from build123d import *

# Parameters (mm, degrees)
CHAMFER1_SIZE  = 3
CHAMFER1_SIZE2 = 0.803847577


with BuildPart() as part:
    # Sketch1 → Revolve1 (revolve)
    with BuildSketch(Plane.XY, mode=Mode.PRIVATE) as revolve1_sk:
        Polygon((42.5, 31), (50, 31), (50, 3), (63.5, 3), (63.5, 0), (67.5, 0), (67.5, -8), (42.5, -8), align=None)
    revolve(revolve1_sk.sketch.rotate(Axis((0, 0, 0), (0, 1, 0)), 90), axis=Axis((0, 0, 0), (0, 1, 0)))

    # Chamfer1
    chamfer1_edges = [part.edges().sort_by_distance(p)[0] for p in [
        (0, 31, 50),
    ]]
    chamfer1_side = [part.faces().sort_by_distance(p)[0] for p in [
        (0, 17, 50),
    ]]
    chamfer(chamfer1_edges, length=CHAMFER1_SIZE, length2=CHAMFER1_SIZE2, reference=chamfer1_side[0])


solid = part.part
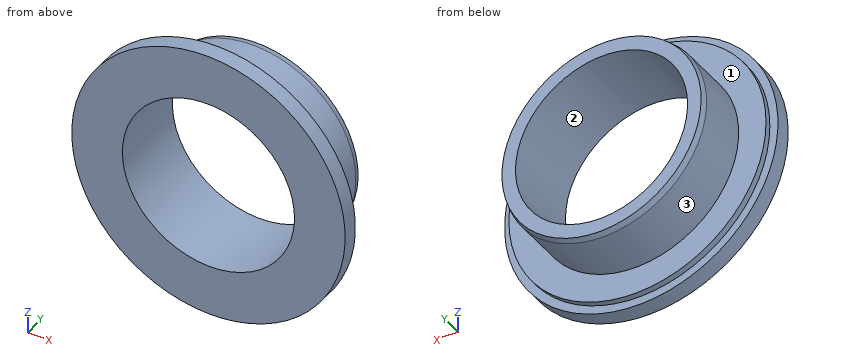
For this review, take the finished solid that the model builds, in its own axes (mm). Face numbers are marked on the shaded views. Round coordinates to 2 decimals unless told otherwise and drop trailing zeros. Loops run counter-clockwise (first coordinate to the right, second up) from the corner with the lowest first, then second, coordinate; pieces in that order, holes last. Notation, with made-up numbers: (-30, 59.5) - (11, 59.5) arc R15 ccw to (11, 85.5) - close; hole circle Ø10 at (46.5, 21.25). An arc over 180 degrees is marked (long way). Answer as CSV lines item,"result".
(1) Consider section A-A on x = 0. Give the boundary of the cut face in (y, z).
Checked values:
outline,"(-8, -67.5) - (0, -67.5) - (0, -63.5) - (3, -63.5) - (3, -50) - (28, -50) - (31, -49.2) - (31, -42.5) - (-8, -42.5) - close; (-8, 42.5) - (31, 42.5) - (31, 49.2) - (28, 50) - (3, 50) - (3, 63.5) - (0, 63.5) - (0, 67.5) - (-8, 67.5) - close"
(2) Mouldability with a two-part tool opening along Z and no side actions: class the marked faces 1, 2 and 3 as +Z half, -Z half, draft (parallel to the pull), parting line (faces both ways), or undercut.
Checked values:
face 1,"draft"
face 2,"undercut"
face 3,"parting line"
(3) Consider section B-B on z = 0. Give the boundary of the cut face in (x, y).
Checked values:
outline,"(-67.5, -8) - (-42.5, -8) - (-42.5, 31) - (-49.2, 31) - (-50, 28) - (-50, 3) - (-63.5, 3) - (-63.5, 0) - (-67.5, 0) - close; (42.5, -8) - (67.5, -8) - (67.5, 0) - (63.5, 0) - (63.5, 3) - (50, 3) - (50, 28) - (49.2, 31) - (42.5, 31) - close"
(4) Insertion check: P1, Ø12, axis at y = 10, z = -21, coming from the -X side; P2, Ø10, axis at x = -49.5, y = 24.5, coming from the -Z side; P3, Ø2, axis at y = 26.5, z = -28.5, coming from the +X side. Each pin has a flat end and moves straight along its axis. Give the tip position at first contact, or say it passes through.
Checked values:
P1,"stops at x = -47.7"
P2,"stops at z = -22.8"
P3,"stops at x = 41.76"
(5) Consider section D-D on y = -3.5. Give the boundary of the cut face in (x, z), then the cut area to 3 significant figures.
Checked values:
outline,"circle Ø135 at (0, 0); hole circle Ø85 at (0, 0)"
area,"8,640 mm2"
(6) Consider section C-C on y = 21. Give the boundary of the cut face in (x, z), then the cut area to 3 significant figures.
Checked values:
outline,"circle Ø100 at (0, 0); hole circle Ø85 at (0, 0)"
area,"2,180 mm2"
(7) Wall thickness on line 1 (X direction, y = 1, z = 0); line 2 (Z direction, x = -0.5, y = -4); line 3 (X direction, y = 16, z = 0): over which ranges is each line inside the solid? List them lowest first.
Checked values:
line 1,"x = -63.5 to -42.5, 42.5 to 63.5"
line 2,"z = -67.5 to -42.5, 42.5 to 67.5"
line 3,"x = -50 to -42.5, 42.5 to 50"
